For this review, take the finished solid that the model builds, in its own axes (mm). Face numbers are marked on the shaded views. A direction names the side the tool comes from. Give positions to 0.01 mm unless a question says otherwise; leave off trailing zeros. Write each loop counter-clockwise with the first axis right and the second up, starting at its lowest first coordinate (ties: lowest second). Pieces come first, ordered by that corner, then holes. Notation, with made-up numbers: M 77.25,41 L 86.25,41 A30 ccw 86.25,78 Z; hole C 40,-4 d11. An arc over 180 degrees is marked long. One line per item, written item: value. Start each with the question number.
Item 1: Consider section A-A, the plane y = 0. Write out the cut boundary in (x, z).
Item 2: Consider section C-C, the plane z = 3.5. Write out the cut boundary in (x, y), and give its area (3 significant figures).
Item 3: Clearance check with flat-ended pins moving along their axes: pin 1 Ø2 at (x, z) = (19, -4) entering from +Y; pin 2 Ø1 at (y, z) = (13.5, -0.5) entering from -X; pin 3 Ø6 at (x, y) = (4, 20.5) entering from -Z; pin 4 Ø2 at (x, z) = (-2, 2) entering from +Y. State where each tip first meets the part, or that it passes through.
Item 4: Consider section D-D, the plane y = 16.5. Write out the cut boundary in (x, z), and give its area (3 significant figures).
Item 5: To check wall thickness, follow probe 1 along Y at (x, z) = (0.5, -4.5); probe 2 along Z at (x, y) = (20.5, 13); probe 3 along X at (y, z) = (-13, 1.5). State the ranges of each line that lie inside material, in increasing order.
Item 6: Tool access review of the marked faces 1 and 2: name each direction out of +Z, -Z, +X, -X, +Y, -Y from which nothing blocks a thin tool from reaching the whole face with its end or side.
Item 7: Mouldability with a two-part tool opening along Y and no side actions: class the marked faces 3, 4 and 5 as released by +Y, released by -Y, zero draft, split by the parting line, or undercut.
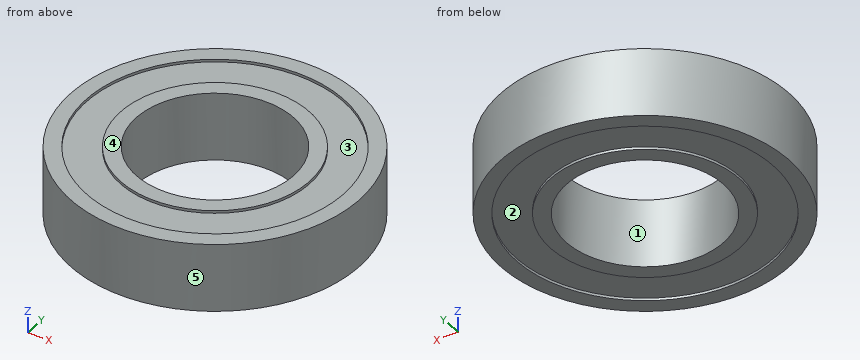
```python
from build123d import *

# Parameters (mm, degrees)
SKETCH1_R           = 27.5
SKETCH1_R_2         = 15
BOSS_EXTRUDE1_DEPTH = 6.5
SKETCH2_R           = 24.5
SKETCH2_R_2         = 18
CUT_EXTRUDE1_DEPTH  = 0.5


with BuildPart() as part:
    # Sketch1 → Boss-Extrude1 (new, symmetric)
    with BuildSketch(Plane.XY):
        with Locations(Location((0, 0, 0), (0, 0, 180))):
            Circle(SKETCH1_R)
        with Locations(Location((0, 0, 0), (0, 0, 180))):
            Circle(SKETCH1_R_2, mode=Mode.SUBTRACT)
    extrude(amount=BOSS_EXTRUDE1_DEPTH, both=True)

    # Sketch2 → Cut-Extrude1 (cut)
    with BuildSketch(Plane.XY.offset(6.5)):
        Circle(SKETCH2_R)
        Circle(SKETCH2_R_2, mode=Mode.SUBTRACT)
    cut_extrude1 = extrude(amount=-CUT_EXTRUDE1_DEPTH, mode=Mode.SUBTRACT)

    # Mirror1: Cut-Extrude1 across plane
    add(cut_extrude1.mirror(Plane.XY), mode=Mode.SUBTRACT)


solid = part.part
```
Model answer:
1. outline: M -27.5,-6.5 L -24.5,-6.5 L -24.5,-6 L -18,-6 L -18,-6.5 L -15,-6.5 L -15,6.5 L -18,6.5 L -18,6 L -24.5,6 L -24.5,6.5 L -27.5,6.5 Z; M 15,-6.5 L 18,-6.5 L 18,-6 L 24.5,-6 L 24.5,-6.5 L 27.5,-6.5 L 27.5,6.5 L 24.5,6.5 L 24.5,6 L 18,6 L 18,6.5 L 15,6.5 Z
2. outline: C 0,0 d55; hole C 0,0 d30
2. area: 1,670 mm2
3. pin 1: stops at y = 20.79
3. pin 2: stops at x = -24.23
3. pin 3: stops at z = -6.5
3. pin 4: stops at y = 27.48
4. outline: M -22,-6.5 L -18.11,-6.5 L -18.11,-6 L -7.19,-6 L -7.19,-6.5 L 7.19,-6.5 L 7.19,-6 L 18.11,-6 L 18.11,-6.5 L 22,-6.5 L 22,6.5 L 18.11,6.5 L 18.11,6 L 7.19,6 L 7.19,6.5 L -7.19,6.5 L -7.19,6 L -18.11,6 L -18.11,6.5 L -22,6.5 Z
4. area: 550 mm2
5. probe 1: y = -27.5 to -14.99, 14.99 to 27.5
5. probe 2: z = -6 to 6
5. probe 3: x = -24.23 to -7.48, 7.48 to 24.23
6. face 1: +Z, -Z
6. face 2: -Z
7. face 3: undercut
7. face 4: zero draft
7. face 5: split by the parting line
